The listing builds one solid part. Answer for the finished solid, in the listing's coordinates (mm). Coordinates: 2 decimals unless noted, no trailing zeros. Order: outer loops, then holes, each group sorted by start corner. A loop starts at its lowest first (then second) coordinate and runs counter-clockwise, first axis right, second up. Notation, with made-up numbers: (-14.5, -28) -> (-9.5, -28) arc R12 cw to (-9.5, -7) -> close; hole circle Ø10 at (86, -14). An arc over 180 degrees is marked (long way). Return JSON: item names as keys, results as strings.
from build123d import *

# Parameters (mm, degrees)
SKETCH1_W           = 60
SKETCH1_H           = 40
SKETCH1_R           = 4.25
SKETCH1_R_2         = 3.3
BOSS_EXTRUDE1_DEPTH = 4
CHAMFER1_SIZE       = 5


with BuildPart() as part:
    # Sketch1 → Boss-Extrude1 (new body)
    with BuildSketch(Plane.XY):
        with Locations((5.009460805, -5.533568905)):
            Rectangle(SKETCH1_W, SKETCH1_H)
        with Locations((-14.990539195, 6.466431095)):
            Circle(SKETCH1_R, mode=Mode.SUBTRACT)
        with Locations((25.009460805, -17.533568905)):
            Circle(SKETCH1_R, mode=Mode.SUBTRACT)
        with Locations((25.009460805, 6.466431095)):
            Circle(SKETCH1_R_2, mode=Mode.SUBTRACT)
        with Locations((-14.990539195, -17.533568905)):
            Circle(SKETCH1_R_2, mode=Mode.SUBTRACT)
    extrude(amount=BOSS_EXTRUDE1_DEPTH)

    # Chamfer1
    chamfer1_edges = [part.edges().sort_by_distance(p)[0] for p in [
        (-24.990539195, 14.466431095, 2),
        (35.009460805, 14.466431095, 2),
        (35.009460805, -25.533568905, 2),
        (-24.990539195, -25.533568905, 2),
    ]]
    chamfer(chamfer1_edges, length=CHAMFER1_SIZE)


solid = part.part
1. The part is cut by section B-B on x = 27. Give the vertices of the cut face in (y, z).
Answer block:
{"outline": "(-25.53, 0) -> (-21.29, 0) -> (-21.29, 4) -> (-25.53, 4) -> close; (-13.78, 0) -> (3.83, 0) -> (3.83, 4) -> (-13.78, 4) -> close; (9.1, 0) -> (14.47, 0) -> (14.47, 4) -> (9.1, 4) -> close"}
2. Determine the mould class of faces 1 (the face through (-18.12, 9.34, 1.97)), 2 (the face through (28.058, 5.203, 1.972)), 3 (the face through (-22.456, -23.069, 1.972)), 4 (the face through (35.009, -6, 2)) for opening direction Y: pulls with the +Y half, pulls with the -Y half, needs draft (parallel to the pull), parting line crosses it, or undercut.
Answer block:
{"face 1": "undercut", "face 2": "undercut", "face 3": "pulls with the -Y half", "face 4": "needs draft"}
3. Consider line 1 (X direction, y = -15.5, z = 2.35); line 2 (Y direction, x = -12, z = 3.2); line 3 (Y direction, x = -20, z = 2). Determine where each line is inside the solid, lowest interval first. Write a range as from..to.
Answer block:
{"line 1": "x = -24.99..-17.59, -12.39..21.28, 28.74..35.01", "line 2": "y = -25.53..-18.93, -16.14..3.45, 9.49..14.47", "line 3": "y = -25.52..14.46"}
4. Each of these flat-tipped pins is pushed along its axis until it touches: pin 1 Ø1 at (x, y) = (-6, -18) entering from -Z; pin 2 Ø4 at (x, y) = (-14.99, -17.53) entering from -Z. Where does it stop, or does it pass through?
Answer block:
{"pin 1": "stops at z = 0", "pin 2": "passes through"}
5. The part is cut by section C-C on z = 3.2. Give the vertices of the cut face in (x, y).
Answer block:
{"outline": "(-24.99, -20.53) -> (-19.99, -25.53) -> (30.01, -25.53) -> (35.01, -20.53) -> (35.01, 9.47) -> (30.01, 14.47) -> (-19.99, 14.47) -> (-24.99, 9.47) -> close; hole circle Ø8.5 at (-14.99, 6.47); hole circle Ø6.6 at (-14.99, -17.53); hole circle Ø8.5 at (25.01, -17.53); hole circle Ø6.6 at (25.01, 6.47)"}
6. The part is cut by section A-A on y = -18.5. Give the vertices of the cut face in (x, z), and give its area (3 significant figures).
Answer block:
{"outline": "(-24.99, 0) -> (-18.15, 0) -> (-18.15, 4) -> (-24.99, 4) -> close; (-11.84, 0) -> (20.87, 0) -> (20.87, 4) -> (-11.84, 4) -> close; (29.15, 0) -> (35.01, 0) -> (35.01, 4) -> (29.15, 4) -> close", "area": "182 mm2"}
